from build123d import *

# Parameters (mm, degrees)
EXTRUDE_1_DEPTH = 140
EXTRUDE_START   = -5
EXTRUDE_2_DEPTH = 5


with BuildPart() as part:
    # 草图1 → 凸台-拉伸1 (new body)
    with BuildSketch(Plane(origin=(0, 0, 0), x_dir=(1, 0, 0), z_dir=(0, 1, 0))):
        with BuildLine():
            Line((-19, -12.278106509), (19, -12.278106509))
            ThreePointArc((19, -12.278106509), (23.242640687, -10.520747196), (25, -6.278106509))
            Line((25, -6.278106509), (25, 31.721893491))
            ThreePointArc((25, 31.721893491), (23.242640687, 35.964534178), (19, 37.721893491))
            Line((19, 37.721893491), (-19, 37.721893491))
            ThreePointArc((-19, 37.721893491), (-23.242640687, 35.964534178), (-25, 31.721893491))
            Line((-25, 31.721893491), (-25, -6.278106509))
            ThreePointArc((-25, -6.278106509), (-23.242640687, -10.520747196), (-19, -12.278106509))
        make_face()
        with BuildLine():
            Line((-19, -7.278106509), (19, -7.278106509))
            ThreePointArc((19, -7.278106509), (19.707106781, -6.98521329), (20, -6.278106509))
            Line((20, -6.278106509), (20, 31.721893491))
            ThreePointArc((20, 31.721893491), (19.707106781, 32.429000272), (19, 32.721893491))
            Line((19, 32.721893491), (-19, 32.721893491))
            ThreePointArc((-19, 32.721893491), (-19.707106781, 32.429000272), (-20, 31.721893491))
            Line((-20, 31.721893491), (-20, -6.278106509))
            ThreePointArc((-20, -6.278106509), (-19.707106781, -6.98521329), (-19, -7.278106509))
        make_face(mode=Mode.SUBTRACT)
    extrude(amount=EXTRUDE_1_DEPTH)

    # 草图2 → 凸台-拉伸2 (add)
    with BuildSketch(Plane(origin=(0, 140, 0), x_dir=(1, 0, 0), z_dir=(0, 1, 0)).offset(EXTRUDE_START)):
        with BuildLine():
            Line((-19, -12.278106509), (19, -12.278106509))
            ThreePointArc((19, -12.278106509), (23.242640687, -10.520747196), (25, -6.278106509))
            Line((25, -6.278106509), (25, 31.721893491))
            ThreePointArc((25, 31.721893491), (23.242640687, 35.964534178), (19, 37.721893491))
            Line((19, 37.721893491), (-19, 37.721893491))
            ThreePointArc((-19, 37.721893491), (-23.242640687, 35.964534178), (-25, 31.721893491))
            Line((-25, 31.721893491), (-25, -6.278106509))
            ThreePointArc((-25, -6.278106509), (-23.242640687, -10.520747196), (-19, -12.278106509))
        make_face()
    extrude(amount=EXTRUDE_2_DEPTH)


solid = part.part
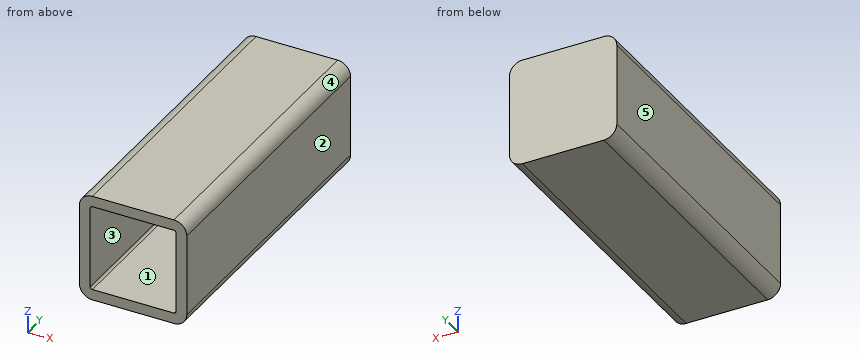
Model file for the job. Use its own axes, mm. Face numbers are marked on the shaded views. A direction names the side the tool comes from. Round coordinates to 2 decimals unless told otherwise and drop trailing zeros. Loops run counter-clockwise (first coordinate to the right, second up) from the corner with the lowest first, then second, coordinate; pieces in that order, holes last. Notation, with made-up numbers: M 79,23 L 128,23 A12 cw 128,28 Z; hole C 7,-30 d11. An arc over 180 degrees is marked long. One line per question, with ' | ' between items.
1) Mould opens along X. For the marked faces 3, 4 and 5 say: +X half, -X half, draft (parallel to the pull), parting line (faces both ways), or undercut.
Solved:
face 3: undercut | face 4: +X half | face 5: -X half
2) Band-saw the part on C-C (x = 14). Give the cut face in (y, z).
Solved:
outline: M 0,-37.72 L 140,-37.72 L 140,12.28 L 0,12.28 L 0,7.28 L 135,7.28 L 135,-32.72 L 0,-32.72 Z
3) Band-saw the part on B-B (z = -18.5). Give the cut face in (x, y), then the cut area to 3 significant figures.
Solved:
outline: M -25,0 L -20,0 L -20,135 L 20,135 L 20,0 L 25,0 L 25,140 L -25,140 Z | area: 1,600 mm²
4) Band-saw the part on A-A (y = 36). Give the cut face in (x, z).
Solved:
outline: M -25,-31.72 A6 ccw -19,-37.72 L 19,-37.72 A6 ccw 25,-31.72 L 25,6.28 A6 ccw 19,12.28 L -19,12.28 A6 ccw -25,6.28 Z; hole M -20,-31.72 A1 ccw -19,-32.72 L 19,-32.72 A1 ccw 20,-31.72 L 20,6.28 A1 ccw 19,7.28 L -19,7.28 A1 ccw -20,6.28 Z
5) Drill centre lines: line 1 along X through (y, z) = (22, 4); line 2 along Z through (x, y) = (13, 59); line 3 along Y through (x, z) = (8, -11.5). Where is each one in solid material? Low to high.
Solved:
line 1: x = -25 to -20, 20 to 25 | line 2: z = -37.72 to -32.72, 7.28 to 12.28 | line 3: y = 135 to 140
6) 3-axis set-ups, long thin cutter, end or side, ignore diameter. For the marked faces 1 and 2: which of +Z, -Z, +X, -X, +Y, -Y reach the whole face in a straight line?
Solved:
face 1: -Y | face 2: +Z, -Z, +X, +Y, -Y
